The model under review builds one solid part; all positions refer to its coordinate system, in mm. Face numbers are marked on the shaded views. A direction names the side the tool comes from. Coordinates: 2 decimals unless noted, no trailing zeros. Write each loop counter-clockwise with the first axis right and the second up, starting at its lowest first coordinate (ties: lowest second). Pieces come first, ordered by that corner, then holes.
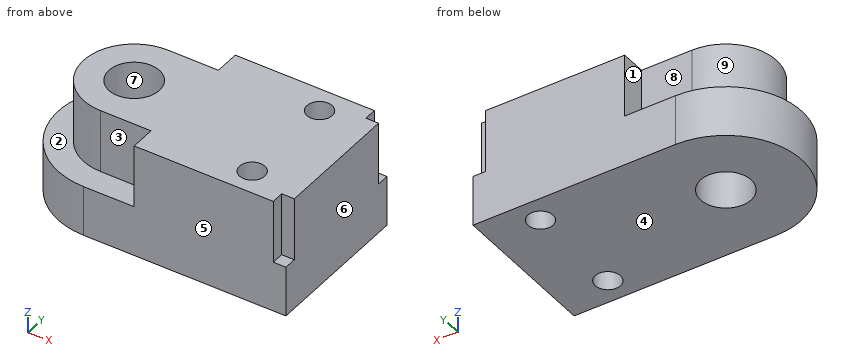
```python
from build123d import *

# Parameters (mm, degrees)
BASE_BLOCK_SKETCH_R       = 10
BASE_BLOCK_DEPTH          = 20
LUG_BOSS_SKETCH_R         = 10
LUG_BOSS_SKETCH_R_2       = 5
LUG_BOSS_WITH_HOLES_DEPTH = 25
SLOT_CUT_SKETCH_R         = 5
SLOT_CUT_DEPTH            = 97.566039579


with BuildPart() as part:
    # Base Block Sketch → Base Block (new body)
    with BuildSketch(Plane.XY):
        with BuildLine():
            Line((0, 30), (80, 30))
            Line((80, 30), (80, -30))
            Line((80, -30), (0, -30))
            ThreePointArc((0, -30), (-30, 0), (0, 30))
        make_face()
        Circle(BASE_BLOCK_SKETCH_R, mode=Mode.SUBTRACT)
    extrude(amount=BASE_BLOCK_DEPTH)

    # Lug Boss Sketch → Lug Boss With Holes (add)
    with BuildSketch(Plane.XY.offset(20)):
        with BuildLine():
            Line((0, 20), (20, 20))
            Line((20, 20), (20, 30))
            Line((20, 30), (75, 30))
            Line((75, 30), (75, 25))
            Line((75, 25), (80, 25))
            Line((80, 25), (80, -25))
            Line((80, -25), (75, -25))
            Line((75, -25), (75, -30))
            Line((75, -30), (20, -30))
            Line((20, -30), (20, -20))
            Line((20, -20), (0, -20))
            ThreePointArc((0, -20), (-20, 0), (0, 20))
        make_face()
        Circle(LUG_BOSS_SKETCH_R, mode=Mode.SUBTRACT)
        with Locations((60, 20)):
            Circle(LUG_BOSS_SKETCH_R_2, mode=Mode.SUBTRACT)
        with Locations((60, -20)):
            Circle(LUG_BOSS_SKETCH_R_2, mode=Mode.SUBTRACT)
    extrude(amount=LUG_BOSS_WITH_HOLES_DEPTH)

    # Slot Cut Sketch → Slot Cut (cut, through all)
    with BuildSketch(Plane.XY.offset(45)):
        with Locations((60, -20)):
            Circle(SLOT_CUT_SKETCH_R)
        with Locations((60, 20)):
            Circle(SLOT_CUT_SKETCH_R)
    extrude(amount=-SLOT_CUT_DEPTH, mode=Mode.SUBTRACT)


solid = part.part
```
Item 1: Take a section at D-D, the plane y = -23.5. Write out the cut boundary in (x, z).
Solved:
outline: (-18.65, 0) - (56.43, 0) - (56.43, 45) - (20, 45) - (20, 20) - (-18.65, 20) - close; (63.57, 0) - (80, 0) - (80, 45) - (63.57, 45) - close
Item 2: For pin 1 (1.5 mm diameter, centred on y = -28, z = 35, fed in from +X); pin 2 (8 mm diameter, centred on y = 10, z = 15.5, fed in from -X); pin 3 (6 mm diameter, centred on x = 5.5, z = 28.5, fed in from -Y), all flat-tipped, find the tip position at first contact; note any pin that passes through.
Solved:
pin 1: stops at x = 75
pin 2: stops at x = -29.39
pin 3: stops at y = -20
Item 3: To check wall thickness, follow line 1 along Y through (x, z) = (60, 35); line 2 along X through (y, z) = (16.5, 5.5); line 3 along Z through (x, y) = (2, 22). State the ranges of each line that lie inside material, in increasing order.
Solved:
line 1: y = -30 to -25, -15 to 15, 25 to 30
line 2: x = -25.05 to 56.43, 63.57 to 80
line 3: z = 0 to 20
Item 4: Take a section at A-A, the plane y = 0. Write out the cut boundary in (x, z), plus the area to 3 significant figures.
Solved:
outline: (-30, 0) - (-10, 0) - (-10, 45) - (-20, 45) - (-20, 20) - (-30, 20) - close; (10, 0) - (80, 0) - (80, 45) - (10, 45) - close
area: 3,800 mm2
Item 5: Take a section at C-C, the plane z = 13. Write out the cut boundary in (x, y).
Solved:
outline: (0, -30) - (80, -30) - (80, 30) - (0, 30) arc R30 ccw to start; hole circle Ø20 at (0, 0); hole circle Ø10 at (60, -20); hole circle Ø10 at (60, 20)
Item 6: Take a section at B-B, the plane x = 60. Write out the cut boundary in (y, z).
Solved:
outline: (-30, 0) - (-25, 0) - (-25, 45) - (-30, 45) - close; (-15, 0) - (15, 0) - (15, 45) - (-15, 45) - close; (25, 0) - (30, 0) - (30, 45) - (25, 45) - close
Item 7: Mouldability with a two-part tool opening along X and no side actions: class the marked faces 6, 7, 8 and 9 as pulls with the +X half, pulls with the -X half, needs draft (parallel to the pull), parting line crosses it, or undercut.
Solved:
face 6: pulls with the +X half
face 7: undercut
face 8: needs draft
face 9: pulls with the -X half
Item 8: Machinability: for the marked faces 1, 2, 3, 4 and 5, which of the approach directions +Z, -Z, +X, -X, +Y, -Y give a long, thin tool a straight path to every point of the face, cutting with its end or side? Answer none if there is none.
Solved:
face 1: +Z, -X, +Y
face 2: +Z, -X
face 3: +Z, -X, -Y
face 4: -Z, +X, -X, +Y, -Y
face 5: +Z, -Z, +X, -X, -Y
